The model under review builds one solid part; all positions refer to its coordinate system, in mm. Face numbers are marked on the shaded views. A direction names the side the tool comes from. Round coordinates to 2 decimals unless told otherwise and drop trailing zeros. Order: outer loops, then holes, each group sorted by start corner. A loop starts at its lowest first (then second) coordinate and runs counter-clockwise, first axis right, second up. Notation, with made-up numbers: (5.25, 7) -> (24.25, 7) arc R27 cw to (24.25, 23) -> close; hole circle Ø2 at (-3, -32). An arc over 180 degrees is marked (long way). Put each result on its own line as item: value. Start each with the question number.
from build123d import *

# Parameters (mm, degrees)
BOSS_EXTRUDE1_DEPTH = 6


with BuildPart() as part:
    # Sketch1 → Boss-Extrude1 (new body)
    with BuildSketch(Plane.XY):
        with BuildLine():
            Line((-6.75, -54), (-6.75, 54))
            ThreePointArc((-6.75, 54), (0, 60.75), (6.75, 54))
            Line((6.75, 54), (6.75, -54))
            ThreePointArc((6.75, -54), (0, -60.75), (-6.75, -54))
        make_face()
        with BuildLine():
            Line((-5.73, -54), (-5.73, 54))
            ThreePointArc((-5.73, 54), (0, 59.73), (5.73, 54))
            Line((5.73, 54), (5.73, -54))
            ThreePointArc((5.73, -54), (0, -59.73), (-5.73, -54))
        make_face(mode=Mode.SUBTRACT)
    extrude(amount=BOSS_EXTRUDE1_DEPTH)


solid = part.part
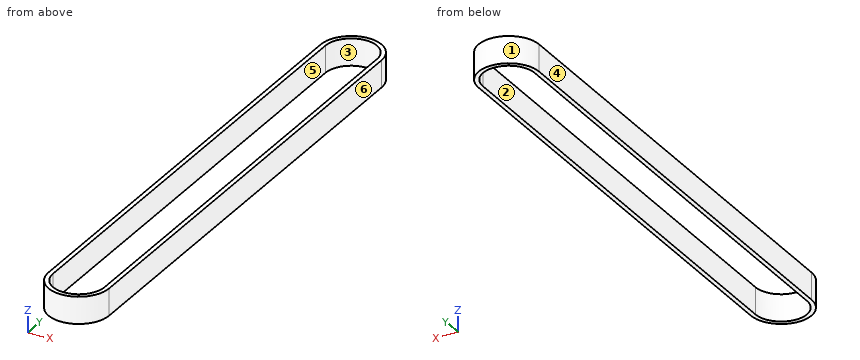
Q1. Draft analysis for pull direction Y (two halves, no side actions). For the marked faces 1, 2, 3 and 4, state which applies: +Y half, -Y half, draft (parallel to the pull), parting line (faces both ways), or undercut.
Q2. Take a section at A-A on x = 0. Give the boundary of the cut face in (y, z), and give its area (3 significant figures).
Q3. Take a section at C-C on z = 4.2. Give the boundary of the cut face in (x, y).
Q4. Wall thickness on probe 1 along X at (y, z) = (22, 4.6); probe 2 along Y at (x, z) = (-0.5, 5.25); probe 3 along Y at (x, z) = (-1.5, 1.05): over which ranges is each line inside the solid? List them lowest first. Write a range as [from, to].
Q5. For the marked faces 5 and 6, list the 3-axis set-ups (+Z, -Z, +X, -X, +Y, -Y) from which the entire face can be reached by the end or side of a thin tool; tool diameter is ignored.
Q6. Clearance check with a flat-ended pin moving along its axis: pin 1 Ø3 at (x, z) = (-4.5, 5) entering from -Y. State where the tip first meets the part, or that it passes through.
Q7. Take a section at B-B on y = -33.5. Give the boundary of the cut face in (x, z), and give its area (3 significant figures).
Calculated:
1. face 1: +Y half
1. face 2: undercut
1. face 3: undercut
1. face 4: draft
2. outline: (-60.75, 0) -> (-59.73, 0) -> (-59.73, 6) -> (-60.75, 6) -> close; (59.73, 0) -> (60.75, 0) -> (60.75, 6) -> (59.73, 6) -> close
2. area: 12.2 mm²
3. outline: (-6.75, -54) arc R6.75 ccw to (6.75, -54) -> (6.75, 54) arc R6.75 ccw to (-6.75, 54) -> close; hole (-5.73, -54) arc R5.73 ccw to (5.73, -54) -> (5.73, 54) arc R5.73 ccw to (-5.73, 54) -> close
4. probe 1: x = [-6.75, -5.73], [5.73, 6.75]
4. probe 2: y = [-60.73, -59.71], [59.71, 60.73]
4. probe 3: y = [-60.58, -59.53], [59.53, 60.58]
5. face 5: +Z, -Z
5. face 6: +Z, -Z, +X, +Y, -Y
6. pin 1: stops at y = -60.05
7. outline: (-6.75, 0) -> (-5.73, 0) -> (-5.73, 6) -> (-6.75, 6) -> close; (5.73, 0) -> (6.75, 0) -> (6.75, 6) -> (5.73, 6) -> close
7. area: 12.2 mm²
